For this review, take the finished solid that the model builds, in its own axes (mm). A direction names the side the tool comes from. Round coordinates to 2 decimals unless told otherwise and drop trailing zeros. Order: outer loops, then holes, each group sorted by start corner. A loop starts at its lowest first (then second) coordinate and runs counter-clockwise, first axis right, second up. Notation, with made-up numbers: M -12,-8 L 23,-8 A13 cw 23,16 Z; hole C 14.25,64.5 d4. An arc over 180 degrees is marked long. Answer as a JSON object with one key per item and string values.
from build123d import *

# Parameters (mm, degrees)
SKETCH1_W          = 33
SKETCH1_H          = 33
EXTRUDE1_DEPTH     = 30
EXTRUDE2_DEPTH     = 16.5
SKETCH4_RX         = 2.5
SKETCH4_RY         = 2.1
CUT_EXTRUDE1_DEPTH = 57.147128155


with BuildPart() as part:
    # Sketch1 → Extrude1 (new body)
    with BuildSketch(Plane.XY):
        Rectangle(SKETCH1_W, SKETCH1_H)
    extrude(amount=EXTRUDE1_DEPTH)

    # Sketch3 → Extrude2 (add, symmetric)
    with BuildSketch(Plane(origin=(0, 0, 0), x_dir=(0, 0, -1), z_dir=(1, 0, 0))):
        Polygon((0, 16.5), (0, -29), (15, -29), (15, -28), (1, -28), (1, 16.5), align=None)
    extrude(amount=EXTRUDE2_DEPTH, both=True)

    # Sketch4 → Cut-Extrude1 (cut, through all)
    with BuildSketch(Plane(origin=(0, -28, 0), x_dir=(1, 0, 0), z_dir=(0, 1, 0))):
        with Locations(Location((-12.5, 8), (0, 0, 90))):
            Ellipse(SKETCH4_RX, SKETCH4_RY)
        with Locations(Location((12.5, 8), (0, 0, -180))):
            Ellipse(SKETCH4_RX, SKETCH4_RY)
    extrude(amount=-CUT_EXTRUDE1_DEPTH, mode=Mode.SUBTRACT)


solid = part.part
1) Machinability: for faces 1 (the flat face through (0, -16.5, 15)), 2 (the flat face through (0, -28, -8)), 3 (the flat face through (0, 16.5, 14)), which of the approach directions +Z, -Z, +X, -X, +Y, -Y give a long, thin tool a straight path to every point of the face, cutting with its end or side? Answer none if there is none.
Geometry check:
{"face 1": "+Z, +X, -X, -Y", "face 2": "-Z, +X, -X, +Y", "face 3": "+Z, -Z, +X, -X, +Y"}
2) Add section C-C on z = -11.5. State the section outline as (x, y) points, and give its area (3 significant figures).
Geometry check:
{"outline": "M -16.5,-29 L 16.5,-29 L 16.5,-28 L -16.5,-28 Z", "area": "33.0 mm²"}
3) Add section B-B on y = 7. State the section outline as (x, z) points, and give its area (3 significant figures).
Geometry check:
{"outline": "M -16.5,-1 L 16.5,-1 L 16.5,30 L -16.5,30 Z", "area": "1,020 mm²"}
4) Insertion check: P1, Ø4, axis at x = 3, y = -24, coming from the +Z side; P2, Ø4, axis at x = 3, z = -7, coming from the +Y side. Each pin has a flat end and moves straight along its axis. Give the tip position at first contact, or say it passes through.
Geometry check:
{"P1": "stops at z = 0", "P2": "stops at y = -28"}
5) Add section A-A on x = 8. State the section outline as (y, z) points.
Geometry check:
{"outline": "M -29,-15 L -28,-15 L -28,-1 L 16.5,-1 L 16.5,30 L -16.5,30 L -16.5,0 L -29,0 Z"}
6) For L1, parallel to Z at x = 10, y = -10; L2, parallel to Y at x = -11, z = 14; L3, parallel to Z at x = 5, y = -21, list the stretches that pass through material, from the lowest coordinate up.
Geometry check:
{"L1": "z = -1 to 30", "L2": "y = -16.5 to 16.5", "L3": "z = -1 to 0"}
